Here's the drawing with two shaded views (mm, measured from the low corner). I have some questions. A direction names the side the tool comes from. Give positions to 0.01 mm unless a question says otherwise; leave off trailing zeros. Loops run counter-clockwise (first coordinate to the right, second up) from the corner with the lowest first, then second, coordinate; pieces in that order, holes last. Notation, with made-up numbers: (-32.5, 84) -> (-20.5, 84) arc R11 ccw to (-20.5, 100) -> close; hole circle Ø10 at (18, 19). An arc over 180 degrees is marked (long way). Answer in a Markdown table with one row per item. Add a question column.
Item 1: If we section it at A-A (x = 30): Write out the boundary of the cut face in (y, z) (3 decimals).
Item 2: If I drill on line 1 (Z direction, x = 30.5, y = 13); line 2 (X direction, y = 6.5, z = 23.5); line 3 (X direction, y = 4.25, z = 44), over which ranges is the centre line in solid material (lowest first)?
Item 3: For P1, Ø4, axis at x = 40.5, y = 5, coming from the -Z side; P2, Ø6, axis at x = 39.5, y = 9.5, coming from the -Z side; P3, Ø1.5, axis at y = 16, z = 40, coming from the -X side, each with a flat end and sliding along its axis, tell me the tip position at first contact or that it passes through.
Item 4: If we section it at C-C (y = 14.75): Write out the boundary of the cut face in (x, z) (3 decimals).
Item 5: If we section it at B-B (z = 30): Write out the boundary of the cut face in (x, y) (3 decimals).
Item 6: We'd pull the mould along X, two halves only. Please class the marked faces 3, 4 and 5: released by +X, released by -X, zero draft, split by the parting line, or undercut.
Item 7: Which directions (+Z, -Z, +X, -X, +Y, -Y) give clear straight access to the entire face, cutting with the end or side of a thin tool? Please do the marked faces 1 and 2.
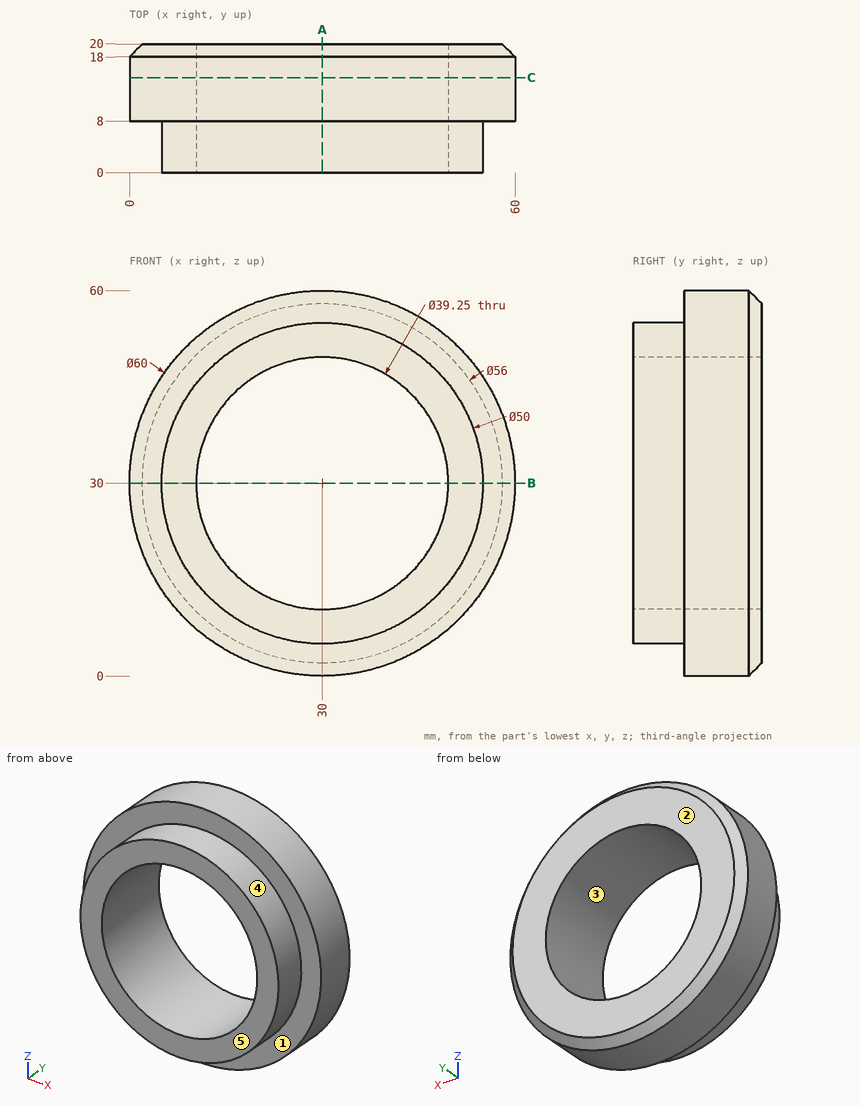
Recorded:
| question | item | result |
|---|---|---|
| 1 | outline | (0, 5) -> (8, 5) -> (8, 0) -> (18, 0) -> (20, 2) -> (20, 10.375) -> (0, 10.375) -> close; (0, 49.625) -> (20, 49.625) -> (20, 58) -> (18, 60) -> (8, 60) -> (8, 55) -> (0, 55) -> close |
| 2 | line 1 | z = 0 to 10.38, 49.62 to 60 |
| 2 | line 2 | x = 5.86 to 11.48, 48.52 to 54.14 |
| 2 | line 3 | x = 9.29 to 16.25, 43.75 to 50.71 |
| 3 | P1 | stops at z = 6.49 |
| 3 | P2 | stops at z = 0.71 |
| 3 | P3 | stops at x = 1.46 |
| 4 | outline | circle Ø60 at (30, 30); hole circle Ø39.25 at (30, 30) |
| 5 | outline | (0, 8) -> (5, 8) -> (5, 0) -> (10.375, 0) -> (10.375, 20) -> (2, 20) -> (0, 18) -> close; (49.625, 0) -> (55, 0) -> (55, 8) -> (60, 8) -> (60, 18) -> (58, 20) -> (49.625, 20) -> close |
| 6 | face 3 | undercut |
| 6 | face 4 | split by the parting line |
| 6 | face 5 | zero draft |
| 7 | face 1 | -Y |
| 7 | face 2 | +Z, -Z, +X, -X, +Y |
